from build123d import *

# Parameters (mm, degrees)
CHAMFER_1_SIZE = 1
CHAMFER_2_SIZE = 1


with BuildPart() as part:
    # 草图1 → 旋转1 (revolve)
    with BuildSketch(Plane.XY, mode=Mode.PRIVATE) as revolve_1_sk:
        Polygon((6.503433875, -2.666983759), (6.503433875, 2.333016241), (8.12324826, 2.333016241), (8.12324826, 17.333016241), (11.713433875, 17.333016241), (11.713433875, -2.666983759), align=None)
    revolve(revolve_1_sk.sketch.rotate(Axis((4.025427808, -22.416983759, 0), (1, 0, 0)), 90), axis=Axis((4.025427808, -22.416983759, 0), (1, 0, 0)))

    # 倒角1
    chamfer_1_edges = [part.edges().sort_by_distance(p)[0] for p in [
        (8.12324826, -22.416983759, -39.75),
    ]]
    chamfer(chamfer_1_edges, length=CHAMFER_1_SIZE)

    # 倒角2
    chamfer_2_edges = [part.edges().sort_by_distance(p)[0] for p in [
        (11.713433875, -22.416983759, -19.75),
    ]]
    chamfer(chamfer_2_edges, length=CHAMFER_2_SIZE)


solid = part.part
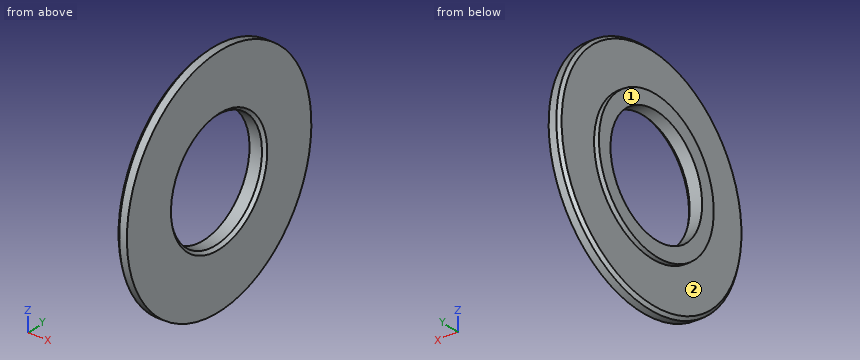
Could you check a few things on this model? Use its own coordinates, in mm. Face numbers are marked on the shaded views. A direction names the side the tool comes from. Give positions to 0.01 mm unless a question says otherwise; leave off trailing zeros. Order: outer loops, then holes, each group sorted by start corner. A loop starts at its lowest first (then second) coordinate and runs counter-clockwise, first axis right, second up. Notation, with made-up numbers: (36, 68) - (84, 68) arc R19 cw to (84, 75) - close; hole circle Ø3 at (63.25, 76.25). An arc over 180 degrees is marked (long way). One line per question, with ' | ' between items. Start each with the question number.
Item 1: For the marked faces 1 and 2, which set-ups out of +Z, -Z, +X, -X, +Y, -Y let a thin tool reach every point of the face, with its end or its side?
Item 2: I want a section at A-A on z = 0. Write out the boundary of the cut face in (x, y).
Item 3: I need wall thicknesses on probe 1 along Y at (x, z) = (8.05, 0); probe 2 along X at (y, z) = (-57.5, 1); probe 3 along Y at (x, z) = (9.9, -17.5). Which ranges of each line are inside material? Lowest first, please. Write a range as [from, to].
Item 4: I'm going to push flat-ended pins straight in: pin 1 Ø3 at (y, z) = (-7, -28) entering from -X; pin 2 Ø3 at (x, y) = (8.5, 5) entering from -Z; pin 3 Ø1 at (x, y) = (9.5, -30) entering from -Z. Where does each tip first touch, or does it pass through?
Verdict:
1) face 1: +Z, -Z, -X, +Y, -Y | face 2: -X
2) outline: (6.5, -47.17) - (8.12, -47.17) - (8.12, -61.17) - (9.12, -62.17) - (11.71, -62.17) - (11.71, -43.17) - (10.71, -42.17) - (6.5, -42.17) - close; (6.5, -2.67) - (10.71, -2.67) - (11.71, -1.67) - (11.71, 17.33) - (9.12, 17.33) - (8.12, 16.33) - (8.12, 2.33) - (6.5, 2.33) - close
3) probe 1: [-47.17, -42.17], [-2.67, 2.33] | probe 2: [8.12, 11.71] | probe 3: [-58.11, -31.57], [-13.26, 13.27]
4) pin 1: x = 8.12 | pin 2: z = -30.02 | pin 3: z = -39.11
